from build123d import *

# Parameters (mm, degrees)
SKETCH1_W           = 40
SKETCH1_H           = 30
BOSS_EXTRUDE1_DEPTH = 12
BOSS_EXTRUDE3_START = 5
BOSS_EXTRUDE3_DEPTH = 5


with BuildPart() as part:
    # Sketch1 → Boss-Extrude1 (new body)
    with BuildSketch(Plane.XY):
        with Locations((20, -15)):
            Rectangle(SKETCH1_W, SKETCH1_H)
    extrude(amount=BOSS_EXTRUDE1_DEPTH)

    # Sketch2 → Boss-Extrude3 (add)
    with BuildSketch(Plane.XY.offset(BOSS_EXTRUDE3_START)):
        Polygon((17.5, 10), (17.5, 2), (5, 0), (35, 0), (22.5, 2), (22.5, 10), align=None)
    extrude(amount=BOSS_EXTRUDE3_DEPTH)


solid = part.part
Model file for the job. Use its own axes, mm. A direction names the side the tool comes from. Coordinates: 2 decimals unless noted, no trailing zeros. Write each loop counter-clockwise with the first axis right and the second up, starting at its lowest first coordinate (ties: lowest second). Pieces come first, ordered by that corner, then holes. Notation, with made-up numbers: (2.25, 45) - (46.25, 45) arc R28 ccw to (46.25, 79) - close; hole circle Ø8 at (4, 59). An arc over 180 degrees is marked (long way). Write each question's results on one line, items separated by ' | '. Start each with the question number.
1) Cut at A-A (x = 27). Write the cut outline in (y, z), then the cut area to 3 significant figures.
2) Flat gauge pins, fed straight in: P1, Ø5, axis at x = 26, y = 7.5, coming from the +Z side; P2, Ø4, axis at y = 7.5, z = 8.5, coming from the +X side. Where does each tip first touch, or does it go through?
3) Probe line 1 along Y through (x, z) = (28, 3.25); line 2 along X through (y, z) = (2.5, 7); line 3 along Y through (x, z) = (6, 8.5). List the from-to ranges inside material, lowest first. Write a range as from..to.
4) Cut at D-D (y = 6.5). Write the cut outline in (x, z).
5) 3-axis set-ups, long thin cutter, end or side, ignore diameter. For faces 1 (the face through (20, 4, 5)), 2 (the face through (20, 4, 10)), 3 (the face through (17.5, 6, 7)), 4 (the face through (22.5, 6, 7)): which of +Z, -Z, +X, -X, +Y, -Y reach the whole face in a straight line?
6) Cut at B-B (x = 15.5). Write the cut outline in (y, z).
7) Cut at C-C (z = 1.25). Write the cut outline in (x, y), then the cut area to 3 significant figures.
Returned:
1) outline: (-30, 0) - (0, 0) - (0, 5) - (1.28, 5) - (1.28, 10) - (0, 10) - (0, 12) - (-30, 12) - close | area: 366 mm^2
2) P1: through | P2: x = 22.5
3) line 1: -30..0 | line 2: 17.5..22.5 | line 3: -30..0.16
4) outline: (17.5, 5) - (22.5, 5) - (22.5, 10) - (17.5, 10) - close
5) face 1: -Z, +X, -X, +Y | face 2: +Z, +X, -X, +Y | face 3: +Z, -Z, -X, +Y | face 4: +Z, -Z, +X, +Y
6) outline: (-30, 0) - (0, 0) - (0, 5) - (1.68, 5) - (1.68, 10) - (0, 10) - (0, 12) - (-30, 12) - close
7) outline: (0, -30) - (40, -30) - (40, 0) - (0, 0) - close | area: 1,200 mm^2
